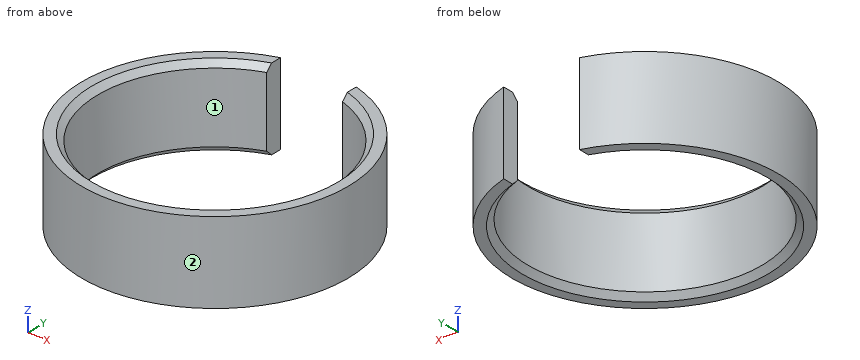
from build123d import *

# Parameters (mm, degrees)
SKETCH1_R           = 11.5
SKETCH1_R_2         = 10.1
BOSS_EXTRUDE1_DEPTH = 7
SKETCH2_W           = 6.5
SKETCH2_H           = 15
CUT_EXTRUDE1_DEPTH  = 18.70593121
CHAMFER1_SIZE       = 0.5


with BuildPart() as part:
    # Sketch1 → Boss-Extrude1 (new body)
    with BuildSketch(Plane.XY):
        Circle(SKETCH1_R)
        Circle(SKETCH1_R_2, mode=Mode.SUBTRACT)
    extrude(amount=BOSS_EXTRUDE1_DEPTH)

    # Sketch2 → Cut-Extrude1 (cut, through all)
    with BuildSketch(Plane.XY.offset(7)):
        with Locations((0, 7.5)):
            Rectangle(SKETCH2_W, SKETCH2_H)
    extrude(amount=-CUT_EXTRUDE1_DEPTH, mode=Mode.SUBTRACT)

    # Chamfer1
    chamfer1_edges = [part.edges().sort_by_distance(p)[0] for p in [
        (0, -10.1, 0),
        (0, -10.1, 7),
    ]]
    chamfer(chamfer1_edges, length=CHAMFER1_SIZE)


solid = part.part
Geometry check sheet. Reference: the model listing, model coordinates, mm. Face numbers are marked on the shaded views. Give positions to 0.01 mm unless a question says otherwise; leave off trailing zeros. Write each loop counter-clockwise with the first axis right and the second up, starting at its lowest first coordinate (ties: lowest second). Pieces come first, ordered by that corner, then holes.
1) Thickness scan on line 1 (X direction, y = 0, z = 3.7); line 2 (Y direction, x = -4, z = 3); line 3 (X direction, y = 6, z = 1.5). Record the ranges inside material, lowest first.
Values follow:
line 1: x = -11.5 to -10.1, 10.1 to 11.5
line 2: y = -10.78 to -9.27, 9.27 to 10.78
line 3: x = -9.81 to -8.12, 8.12 to 9.81
2) Go/stop test with flat-tipped pins: pin 1 Ø2 at (x, z) = (-4, 2) entering from -Y; pin 2 Ø4 at (x, z) = (8, 5) entering from -Y; pin 3 Ø1 at (x, y) = (-1, 8.5) entering from -Z; pin 4 Ø1.2 at (y, z) = (10, 3.5) entering from -X. Record where each tip stops, or that it passes through.
Values follow:
pin 1: stops at y = -11.1
pin 2: stops at y = -9.81
pin 3: passes through
pin 4: stops at x = -6.62
3) Release check for a two-part mould opening along X. For the marked faces 1 and 2 record: released by +X, released by -X, zero draft, split by the parting line, or undercut.
Values follow:
face 1: undercut
face 2: split by the parting line
4) Cross-section at C-C (z = 6). Record the boundary of the cut face in (x, y).
Values follow:
outline: (-3.25, 9.56) - (-3.25, 11.03) arc R11.5 ccw (long way) to (3.25, 11.03) - (3.25, 9.56) arc R10.1 cw (long way) to start
5) Cross-section at A-A (y = 0). Record the boundary of the cut face in (x, z), plus the area to 3 significant figures.
Values follow:
outline: (-11.5, 0) - (-10.6, 0) - (-10.1, 0.5) - (-10.1, 6.5) - (-10.6, 7) - (-11.5, 7) - close; (10.1, 0.5) - (10.6, 0) - (11.5, 0) - (11.5, 7) - (10.6, 7) - (10.1, 6.5) - close
area: 19.1 mm2
6) Cross-section at B-B (x = 0). Record the boundary of the cut face in (y, z).
Values follow:
outline: (-11.5, 0) - (-10.6, 0) - (-10.1, 0.5) - (-10.1, 6.5) - (-10.6, 7) - (-11.5, 7) - close
